```python
from build123d import *

# Parameters (mm, degrees)
BLOCK_PROFILE_SKETCH_W         = 65
BLOCK_PROFILE_SKETCH_H         = 41
BLOCK_PROFILE_SKETCH_R         = 5
BLOCK_BODY_80MM_DEPTH          = 40
EDGE_CHAMFER_5MM_SIZE          = 5
TOP_CHAMFER_21MM_X_35DEG_SIZE  = 21
TOP_CHAMFER_21MM_X_35DEG_SIZE2 = 14.704358302
TOP_RECESS_CUT_6MM_DEPTH       = 6
LUG_GAP_CUT_60MM_DEPTH         = 60
THROUGH_SLOT_SKETCH_W          = 5
THROUGH_SLOT_SKETCH_H          = 22
THROUGH_SLOT_CUT_DEPTH         = 210


with BuildPart() as part:
    # Block Profile Sketch → Block Body 80mm (new, symmetric)
    with BuildSketch(Plane.XY):
        with Locations((32.5, 20.5)):
            Rectangle(BLOCK_PROFILE_SKETCH_W, BLOCK_PROFILE_SKETCH_H)
        with Locations((12, 31)):
            Circle(BLOCK_PROFILE_SKETCH_R, mode=Mode.SUBTRACT)
    extrude(amount=BLOCK_BODY_80MM_DEPTH, both=True)

    # Edge Chamfer 5mm
    edge_chamfer_5mm_edges = [part.edges().sort_by_distance(p)[0] for p in [
        (0, 41, 0),
    ]]
    chamfer(edge_chamfer_5mm_edges, length=EDGE_CHAMFER_5MM_SIZE)

    # Top Chamfer 21mm x 35deg
    top_chamfer_21mm_x_35deg_edges = [part.edges().sort_by_distance(p)[0] for p in [
        (65, 41, 0),
    ]]
    top_chamfer_21mm_x_35deg_side = [part.faces().sort_by_distance(p)[0] for p in [
        (35, 41, 0),
    ]]
    chamfer(top_chamfer_21mm_x_35deg_edges, length=TOP_CHAMFER_21MM_X_35DEG_SIZE, length2=TOP_CHAMFER_21MM_X_35DEG_SIZE2, reference=top_chamfer_21mm_x_35deg_side[0])

    # Top Recess Sketch → Top Recess Cut 6mm (cut)
    with BuildSketch(Plane.XY.offset(40)):
        with BuildLine():
            Line((0, 13), (14.264629746, 13))
            ThreePointArc((14.264629746, 13), (34.056650789, 21.881854304), (49.396602602, 37.221258177))
            Line((49.396602602, 37.221258177), (44, 41))
            Line((44, 41), (5, 41))
            Line((5, 41), (0, 36))
            Line((0, 36), (0, 13))
        make_face()
    extrude(amount=-TOP_RECESS_CUT_6MM_DEPTH, mode=Mode.SUBTRACT)

    # Lug Gap Sketch → Lug Gap Cut 60mm (cut)
    with BuildSketch(Plane.XY.offset(30)):
        with BuildLine():
            Line((0, 13), (0, 36))
            Line((0, 36), (5, 41))
            Line((5, 41), (44, 41))
            Line((44, 41), (49.396602602, 37.221258177))
            ThreePointArc((49.396602602, 37.221258177), (34.056650789, 21.881854304), (14.264629746, 13))
            Line((14.264629746, 13), (0, 13))
        make_face()
    extrude(amount=-LUG_GAP_CUT_60MM_DEPTH, mode=Mode.SUBTRACT)

    # Through Slot Sketch → Through Slot Cut (cut)
    with BuildSketch(Plane(origin=(0, 41, 0), x_dir=(1, 0, 0), z_dir=(0, 1, 0))):
        with Locations((62.5, 0)):
            Rectangle(THROUGH_SLOT_SKETCH_W, THROUGH_SLOT_SKETCH_H)
    extrude(amount=-THROUGH_SLOT_CUT_DEPTH, mode=Mode.SUBTRACT)


solid = part.part
```
For this review, take the finished solid that the model builds, in its own axes (mm). A direction names the side the tool comes from. Coordinates: 2 decimals unless noted, no trailing zeros. Write each loop counter-clockwise with the first axis right and the second up, starting at its lowest first coordinate (ties: lowest second). Pieces come first, ordered by that corner, then holes.
(1) For pin 1 Ø6 at (x, z) = (42, 19) entering from -Y; pin 2 Ø1.8 at (x, z) = (7, 37.5) entering from +Y; pin 3 Ø17.5 at (y, z) = (17, 2) entering from +X; pin 4 Ø6 at (x, z) = (50.5, 7.5) entering from +Y, all flat-tipped, find the tip position at first contact; note any pin that passes through.
(2) The part is to be moulded in two halves that separate along Y. For faces 4 (the face through (16.619, 29.085, -35.07)), 5 (the face through (39, 11, 40)), 6 (the face through (24, 41, 32)), 7 (the face through (16.619, 29.085, 31.972)), say which applies: +Y half, -Y half, draft (parallel to the pull), parting line (faces both ways), or undercut.
(3) Add section B-B on y = 31. Give the boundary of the cut face in (x, z).
(4) Add section D-D on y = 10. Give the boundary of the cut face in (x, z).
(5) Wall thickness on probe 1 along Y at (x, z) = (12, -34.5); probe 2 along Z at (x, y) = (9.5, 39); probe 3 along X at (y, z) = (3.5, -5): over which ranges is each line inside the solid? List them lowest first.
(6) Tool access review of faces 1 (the face through (24, 41, -35)), 2 (the face through (20, 27, 30)), 3 (the face through (33.805, 21.709, 37.042)): name each direction out of +Z, -Z, +X, -X, +Y, -Y from which nothing blocks a thin tool from reaching the whole face with its end or side.
(7) Add section A-A on x = 12. Give the boundary of the cut face in (y, z), then the cut area to 3 significant figures.
(8) Add section C-C on z = 27. Give the boundary of the cut face in (x, y), then the cut area to 3 significant figures.
Answer sheet:
1. pin 1: stops at y = 0
1. pin 2: stops at y = 13
1. pin 3: stops at x = 60
1. pin 4: stops at y = 37.22
2. face 4: undercut
2. face 5: draft
2. face 6: +Y half
2. face 7: undercut
3. outline: (0, -40) - (7, -40) - (7, -30) - (0, -30) - close; (0, 30) - (7, 30) - (7, 34) - (0, 34) - close; (17, -40) - (58.28, -40) - (58.28, 40) - (44.47, 40) - (44.47, 34) - (17, 34) - (17, 30) - (44.47, 30) - (44.47, -30) - (17, -30) - close
4. outline: (0, -40) - (65, -40) - (65, -11) - (60, -11) - (60, 11) - (65, 11) - (65, 40) - (0, 40) - close
5. probe 1: y = 0 to 26, 36 to 41
5. probe 2: z = -40 to -30, 30 to 34
5. probe 3: x = 0 to 60
6. face 1: +Z, -Z, +X, -X, +Y
6. face 2: -X, +Y
6. face 3: +Z, -X, +Y
7. outline: (0, -40) - (26, -40) - (26, -30) - (13, -30) - (13, 30) - (26, 30) - (26, 34) - (13, 34) - (13, 40) - (0, 40) - close; (36, -40) - (41, -40) - (41, -30) - (36, -30) - close; (36, 30) - (41, 30) - (41, 34) - (36, 34) - close
7. area: 1,290 mm2
8. outline: (0, 0) - (65, 0) - (65, 26.3) - (49.4, 37.22) arc R60 cw to (14.26, 13) - (0, 13) - close
8. area: 1,450 mm2
